```python
from build123d import *

# Parameters (mm, degrees)
EXTRUDE_1_DEPTH     = 15
SKETCH_2_R          = 2
CUT_EXTRUDE_1_DEPTH = 15
FILLET_1_R          = 3


with BuildPart() as part:
    # 草图1 → 凸台-拉伸1 (new body)
    with BuildSketch(Plane.XY):
        Polygon((0, 0), (15, 0), (15, 15), (105, 15), (105, 0), (120, 0), (120, 5), (110, 5), (110, 20), (10, 20), (10, 5), (0, 5), align=None)
    extrude(amount=EXTRUDE_1_DEPTH)

    # 草图2 → 切除-拉伸1 (cut)
    with BuildSketch(Plane(origin=(0, 5, 0), x_dir=(1, 0, 0), z_dir=(0, 1, 0))):
        with Locations(Location((5, -7.5, 0), (0, 0, 270))):
            Circle(SKETCH_2_R)
        with Locations(Location((115, -7.5, 0), (0, 0, 270))):
            Circle(SKETCH_2_R)
    extrude(amount=-CUT_EXTRUDE_1_DEPTH, mode=Mode.SUBTRACT)

    # 圆角1
    fillet_1_edges = [part.edges().sort_by_distance(p)[0] for p in [
        (10, 20, 7.5),
        (110, 20, 7.5),
        (105, 15, 7.5),
        (15, 15, 7.5),
    ]]
    fillet(fillet_1_edges, radius=FILLET_1_R)


solid = part.part
```
Part model, mm, in its own coordinate system. A direction names the side the tool comes from. Round coordinates to 2 decimals unless told otherwise and drop trailing zeros. Order: outer loops, then holes, each group sorted by start corner. A loop starts at its lowest first (then second) coordinate and runs counter-clockwise, first axis right, second up. Notation, with made-up numbers: M -22,85 L 17,85 A30 ccw 17,119 Z; hole C 87.5,48 d9. An arc over 180 degrees is marked long. Put each result on its own line as item: value. Start each with the question number.
1. Slice it at C-C on x = 115. List the corners of the cut face in (y, z), then the cut area to 3 significant figures.
2. Tool access for faces 1 (the face through (116.686, 2.535, 8.575)), 2 (the face through (105, 6, 7)), 3 (the face through (110, 11, 7)), 4 (the face through (10, 11, 7)): list every direction of +Z, -Z, +X, -X, +Y, -Y with a clear straight run to the whole face (end or side of a thin tool).
3. Slice it at A-A on y = 1.5. List the corners of the cut face in (x, z).
4. Slice it at B-B on z = 7.5. List the corners of the cut face in (x, y).
5. Slice it at D-D on y = 8.25. List the corners of the cut face in (x, z), then the cut area to 3 significant figures.
6. Drop flat-ended pins along their axis: pin 1 (6 mm diameter, centred on y = 9, z = 4, fed in from +X); pin 2 (1 mm diameter, centred on x = 35.5, z = 10.5, fed in from -Y); pin 3 (3 mm diameter, centred on x = 69.5, y = 13, fed in from +Z); pin 4 (3.5 mm diameter, centred on y = 12.5, z = 4.5, fed in from -X). Give the stop position or say it passes through.
7. Two-plate mould, pull along X, no slides. Class faces 5 (the face through (5.088, 2.535, 5.502)), 6 (the face through (6.2, 5, 5.7)), 7 (the face through (10.9, 19.14, 7.6)): +X half, -X half, draft (parallel to the pull), parting line (faces both ways), or undercut.
8. Drill centre lines: probe 1 along X at (y, z) = (3.55, 7.5); probe 2 along X at (y, z) = (8.25, 13.5); probe 3 along X at (y, z) = (4, 5.25). Where is each one in solid material? Low to high. Write a range as [from, to].
Findings:
1. outline: M 0,0 L 5,0 L 5,5.5 L 0,5.5 Z; M 0,9.5 L 5,9.5 L 5,15 L 0,15 Z
1. area: 55.0 mm2
2. face 1: +Y, -Y
2. face 2: +Z, -Z, -Y
2. face 3: +Z, -Z, +X, +Y
2. face 4: +Z, -Z, -X, +Y
3. outline: M 0,0 L 15,0 L 15,15 L 0,15 Z; M 105,0 L 120,0 L 120,15 L 105,15 Z; hole C 5,7.5 d4; hole C 115,7.5 d4
4. outline: M 0,0 L 3,0 L 3,5 L 0,5 Z; M 7,0 L 15,0 L 15,12 A3 cw 18,15 L 102,15 A3 cw 105,12 L 105,0 L 113,0 L 113,5 L 110,5 L 110,17 A3 ccw 107,20 L 13,20 A3 ccw 10,17 L 10,5 L 7,5 Z; M 117,0 L 120,0 L 120,5 L 117,5 Z
5. outline: M 10,0 L 15,0 L 15,15 L 10,15 Z; M 105,0 L 110,0 L 110,15 L 105,15 Z
5. area: 150 mm2
6. pin 1: x = 110
6. pin 2: y = 15
6. pin 3: through
6. pin 4: x = 10
7. face 5: undercut
7. face 6: draft
7. face 7: -X half
8. probe 1: [0, 3], [7, 15], [105, 113], [117, 120]
8. probe 2: [10, 15], [105, 110]
8. probe 3: [0, 15], [105, 120]
